For this review, take the finished solid that the model builds, in its own axes (mm). Face numbers are marked on the shaded views. A direction names the side the tool comes from. Round coordinates to 2 decimals unless told otherwise and drop trailing zeros. Order: outer loops, then holes, each group sorted by start corner. A loop starts at its lowest first (then second) coordinate and runs counter-clockwise, first axis right, second up.
```python
from build123d import *

# Parameters (mm, degrees)
BOSS_EXTRUDE1_DEPTH = 10
M4_TAPPED_HOLE1_D   = 3.3
CUT_EXTRUDE1_START  = -30
SKETCH4_R           = 2.55
CUT_EXTRUDE1_DEPTH  = 84
SCALE_FACTOR1_SCALE = 0.7


with BuildPart() as part:
    # Sketch1 → Boss-Extrude1 (new body)
    with BuildSketch(Plane(origin=(0, 0, 0), x_dir=(1, 0, 0), z_dir=(0, 1, 0))):
        with BuildLine():
            Line((-50, -25), (-40, -25))
            ThreePointArc((-40, -25), (-35, -20), (-30, -25))
            Line((-30, -25), (-15, -25))
            ThreePointArc((-15, -25), (-10, -20), (-5, -25))
            Line((-5, -25), (5, -25))
            ThreePointArc((5, -25), (10, -20), (15, -25))
            Line((15, -25), (30, -25))
            ThreePointArc((30, -25), (35, -20), (40, -25))
            Line((40, -25), (50, -25))
            Line((50, -25), (50, 25))
            Line((50, 25), (40, 25))
            ThreePointArc((40, 25), (35, 20), (30, 25))
            Line((30, 25), (15, 25))
            ThreePointArc((15, 25), (10, 20), (5, 25))
            Line((5, 25), (-5, 25))
            ThreePointArc((-5, 25), (-10, 20), (-15, 25))
            Line((-15, 25), (-30, 25))
            ThreePointArc((-30, 25), (-35, 20), (-40, 25))
            Line((-40, 25), (-50, 25))
            Line((-50, 25), (-50, -25))
        make_face()
        with BuildLine():
            Line((-40, 14), (-40, 2))
            Line((-40, 2), (-42, 0))
            Line((-42, 0), (-40, -2))
            Line((-40, -2), (-40, -14))
            ThreePointArc((-40, -14), (-35, -19), (-30, -14))
            Line((-30, -14), (-15, -14))
            ThreePointArc((-15, -14), (-10, -19), (-5, -14))
            Line((-5, -14), (5, -14))
            ThreePointArc((5, -14), (10, -19), (15, -14))
            Line((15, -14), (30, -14))
            ThreePointArc((30, -14), (35, -19), (40, -14))
            Line((40, -14), (40, 14))
            ThreePointArc((40, 14), (35, 19), (30, 14))
            Line((30, 14), (15, 14))
            ThreePointArc((15, 14), (10, 19), (5, 14))
            Line((5, 14), (0, 14))
            Line((0, 14), (-5, 14))
            ThreePointArc((-5, 14), (-10, 19), (-15, 14))
            Line((-15, 14), (-30, 14))
            ThreePointArc((-30, 14), (-35, 19), (-40, 14))
        make_face(mode=Mode.SUBTRACT)
    extrude(amount=BOSS_EXTRUDE1_DEPTH)

    # M4 Tapped Hole1 (through all)
    with Locations(Plane(origin=(0, 0, -25), x_dir=(-1, 0, 0), z_dir=(0, 0, -1))):
        with Locations((0, 5)):
            Hole(M4_TAPPED_HOLE1_D / 2)

    # Sketch4 → Cut-Extrude1 (cut)
    with BuildSketch(Plane.ZY.offset(50).offset(CUT_EXTRUDE1_START)):
        with Locations((0, 5)):
            Circle(SKETCH4_R)
    extrude(amount=-CUT_EXTRUDE1_DEPTH, mode=Mode.SUBTRACT)


with BuildPart() as part_1:
    # Scale factor1: scaled about (0, 0, 0)
    add(part.part.scale(SCALE_FACTOR1_SCALE))


solid = part_1.part
```
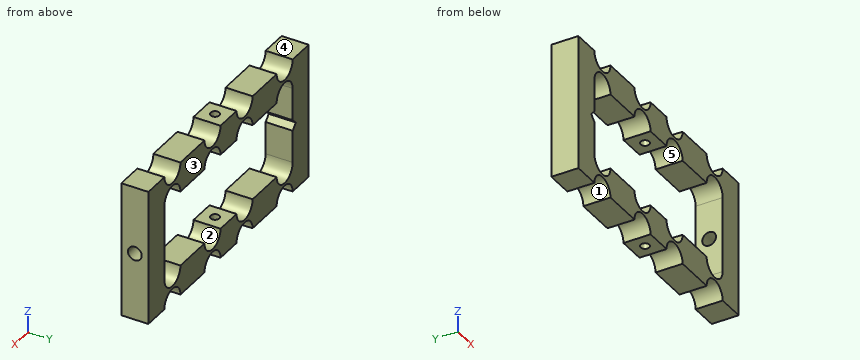
Q1. Take a section at D-D, the plane x = -26. State the section outline as (y, z) points, plus the area to 3 significant figures.
Q2. Clearance check with flat-ended pins moving along their axes: pin 1 (1.5 mm diameter, centred on x = 24, y = 3.5, fed in from -Z); pin 2 (8 mm diameter, centred on x = -6, z = -4, fed in from +Y). State where each tip first meets the part, or that it passes through.
Q3. Mouldability with a two-part tool opening along Z and no side actions: class the marked faces 1, 2 and 3 as +Z half, -Z half, draft (parallel to the pull), parting line (faces both ways), or undercut.
Q4. Take a section at A-A, the plane x = 24.5. State the section outline as (y, z) points, plus the area to 3 significant figures.
Q5. Take a section at B-B, the plane x = 0. State the section outline as (y, z) points (3 decimals).
Q6. Tool access review of the marked faces 4 and 5: name each direction out of +Z, -Z, +X, -X, +Y, -Y from which nothing blocks a thin tool from reaching the whole face with its end or side.
Q7. Wall thickness on line 1 (Z direction, x = 20, y = 4.5); line 2 (Y direction, x = 0, z = 13.25) (3 decimals); line 3 (X direction, y = 3.5, z = 2): over which ranges is each line inside the solid? List them lowest first.
Q8. Take a section at C-C, the plane y = 3.5. Count the separate pieces of the cut face and the enclosed holes in it, plus the area to 3 significant figures.
Working result:
1. outline: (0, -14.34) - (7, -14.34) - (7, -12.96) - (0, -12.96) - close; (0, 12.96) - (7, 12.96) - (7, 14.34) - (0, 14.34) - close
1. area: 19.3 mm2
2. pin 1: stops at z = -14.23
2. pin 2: passes through
3. face 1: -Z half
3. face 2: undercut
3. face 3: draft
4. outline: (0, -14) - (7, -14) - (7, -13.3) - (0, -13.3) - close; (0, 13.3) - (7, 13.3) - (7, 14) - (0, 14) - close
4. area: 9.80 mm2
5. outline: (0, -17.5) - (2.345, -17.5) - (2.345, -9.8) - (0, -9.8) - close; (0, 9.8) - (2.345, 9.8) - (2.345, 17.5) - (0, 17.5) - close; (4.655, -17.5) - (7, -17.5) - (7, -9.8) - (4.655, -9.8) - close; (4.655, 9.8) - (7, 9.8) - (7, 17.5) - (4.655, 17.5) - close
6. face 4: +Z, +X, -X, +Y, -Y
6. face 5: +Y, -Y
7. line 1: z = -17.5 to -9.8, 9.8 to 17.5
7. line 2: y = 0 to 2.345, 4.655 to 7
7. line 3: x = -35 to -28, 28 to 35
8. separate pieces: 3
8. enclosed holes: 0
8. area: 982 mm2
